from build123d import *

# Parameters (mm, degrees)
FLANGE_PLATE_DEPTH        = 25
BOLT_HOLES_SKETCH_R       = 8
BOLT_HOLES_6X_16_DEPTH    = 25
ANNULAR_RECESS_92_DEPTH   = 15
LUG_HOLES_SKETCH_R        = 7
LUG_HOLES_2X_14_DEPTH     = 111.034083526
KEYED_CENTRE_HUB_40_DEPTH = 15


with BuildPart() as part:
    # Flange Profile Sketch → Flange Plate (new body)
    with BuildSketch(Plane(origin=(0, 0, 0), x_dir=(1, 0, 0), z_dir=(0, 1, 0))):
        with BuildLine():
            ThreePointArc((-14.89981335, 63.269230769), (-32.5, 56.291651246), (-47.342854449, 44.538232258))
            ThreePointArc((-47.342854449, 44.538232258), (-69.282032303, 40), (-62.242667799, 18.730998512))
            ThreePointArc((-62.242667799, 18.730998512), (-65, 0), (-62.242667799, -18.730998512))
            ThreePointArc((-62.242667799, -18.730998512), (-69.282032303, -40), (-47.342854449, -44.538232258))
            ThreePointArc((-47.342854449, -44.538232258), (-32.5, -56.291651246), (-14.89981335, -63.269230769))
            ThreePointArc((-14.89981335, -63.269230769), (0, -80), (14.89981335, -63.269230769))
            ThreePointArc((14.89981335, -63.269230769), (32.5, -56.291651246), (47.342854449, -44.538232258))
            ThreePointArc((47.342854449, -44.538232258), (69.282032303, -40), (62.242667799, -18.730998512))
            ThreePointArc((62.242667799, -18.730998512), (65, 0), (62.242667799, 18.730998512))
            ThreePointArc((62.242667799, 18.730998512), (69.282032303, 40), (47.342854449, 44.538232258))
            ThreePointArc((47.342854449, 44.538232258), (32.5, 56.291651246), (14.89981335, 63.269230769))
            ThreePointArc((14.89981335, 63.269230769), (0, 80), (-14.89981335, 63.269230769))
        make_face()
    extrude(amount=FLANGE_PLATE_DEPTH)

    # Bolt Holes Sketch → Bolt Holes 6xØ16 (cut)
    with BuildSketch(Plane(origin=(0, 25, 0), x_dir=(1, 0, 0), z_dir=(0, 1, 0))):
        with Locations(Location((0, 65, 0), (0, 0, 270))):
            Circle(BOLT_HOLES_SKETCH_R)
        with Locations(Location((56.291651246, 32.5, 0), (0, 0, 270))):
            Circle(BOLT_HOLES_SKETCH_R)
        with Locations(Location((56.291651246, -32.5, 0), (0, 0, 270))):
            Circle(BOLT_HOLES_SKETCH_R)
        with Locations(Location((0, -65, 0), (0, 0, 270))):
            Circle(BOLT_HOLES_SKETCH_R)
        with Locations(Location((-56.291651246, -32.5, 0), (0, 0, 270))):
            Circle(BOLT_HOLES_SKETCH_R)
        with Locations(Location((-56.291651246, 32.5, 0), (0, 0, 270))):
            Circle(BOLT_HOLES_SKETCH_R)
    extrude(amount=-BOLT_HOLES_6X_16_DEPTH, mode=Mode.SUBTRACT)

    # Recess Sketch → Annular Recess Ø92 (cut)
    with BuildSketch(Plane(origin=(0, 25, 0), x_dir=(1, 0, 0), z_dir=(0, 1, 0))):
        with BuildLine():
            ThreePointArc((-43.217391304, -15.756176213), (0, -46), (43.217391304, -15.756176213))
            ThreePointArc((43.217391304, -15.756176213), (30, 0), (43.217391304, 15.756176213))
            ThreePointArc((43.217391304, 15.756176213), (0, 46), (-43.217391304, 15.756176213))
            ThreePointArc((-43.217391304, 15.756176213), (-30, 0), (-43.217391304, -15.756176213))
        make_face()
    extrude(amount=-ANNULAR_RECESS_92_DEPTH, mode=Mode.SUBTRACT)

    # Lug Holes Sketch → Lug Holes 2xØ14 (cut, through all)
    with BuildSketch(Plane(origin=(0, 25, 0), x_dir=(1, 0, 0), z_dir=(0, 1, 0))):
        with Locations(Location((-46, 0, 0), (0, 0, 270))):
            Circle(LUG_HOLES_SKETCH_R)
        with Locations(Location((46, 0, 0), (0, 0, 270))):
            Circle(LUG_HOLES_SKETCH_R)
    extrude(amount=-LUG_HOLES_2X_14_DEPTH, mode=Mode.SUBTRACT)

    # Centre Hub Sketch → Keyed Centre Hub Ø40 (add)
    with BuildSketch(Plane(origin=(0, 10, 0), x_dir=(1, 0, 0), z_dir=(0, 1, 0))):
        with BuildLine():
            Line((17.207997686, -10.192390085), (27.532796297, -16.307824137))
            ThreePointArc((27.532796297, -16.307824137), (22.581559349, -22.673181898), (16.196205348, -27.598603811))
            Line((16.196205348, -27.598603811), (10.122628343, -17.249127382))
            ThreePointArc((10.122628343, -17.249127382), (-0.040491828, -19.99995901), (-10.192390085, -17.207997686))
            Line((-10.192390085, -17.207997686), (-16.307824137, -27.532796297))
            ThreePointArc((-16.307824137, -27.532796297), (-22.673181898, -22.581559349), (-27.598603811, -16.196205348))
            Line((-27.598603811, -16.196205348), (-17.249127382, -10.122628343))
            ThreePointArc((-17.249127382, -10.122628343), (-19.99995901, 0.040491828), (-17.207997686, 10.192390085))
            Line((-17.207997686, 10.192390085), (-27.532796297, 16.307824137))
            ThreePointArc((-27.532796297, 16.307824137), (-22.581559349, 22.673181898), (-16.196205348, 27.598603811))
            Line((-16.196205348, 27.598603811), (-10.122628343, 17.249127382))
            ThreePointArc((-10.122628343, 17.249127382), (0.040491828, 19.99995901), (10.192390085, 17.207997686))
            Line((10.192390085, 17.207997686), (16.307824137, 27.532796297))
            ThreePointArc((16.307824137, 27.532796297), (22.673181898, 22.581559349), (27.598603811, 16.196205348))
            Line((27.598603811, 16.196205348), (17.249127382, 10.122628343))
            ThreePointArc((17.249127382, 10.122628343), (19.99995901, -0.040491828), (17.207997686, -10.192390085))
        make_face()
    extrude(amount=KEYED_CENTRE_HUB_40_DEPTH)


solid = part.part
CAD build for the part. Positions are in the model's coordinates, mm. A direction names the side the tool comes from. Coordinates: 2 decimals unless noted, no trailing zeros. Loops run counter-clockwise (first coordinate to the right, second up) from the corner with the lowest first, then second, coordinate; pieces in that order, holes last. Notation, with made-up numbers: (38, 55.5) -> (60, 55.5) arc R9 cw to (60, 66.5) -> close; hole circle Ø7 at (0, 9). An arc over 180 degrees is marked (long way). One line per item, written item: value.
1. Slice it at C-C on z = 65. Write the cut outline in (x, y), and give its area (3 significant figures).
Answers:
outline: (-15, 0) -> (-8, 0) -> (-8, 25) -> (-15, 25) -> close; (8, 0) -> (15, 0) -> (15, 25) -> (8, 25) -> close
area: 350 mm^2
2. Pull direction X, two halves, no side cores. Call faces 3 (the face through (0, 12, 80)), 4 (the face through (65, 12, 0)), 5 (the face through (69.101, 12.325, 40.305)), 6 (the face through (31, 25, -1)): pulls with the +X half, pulls with the -X half, needs draft (parallel to the pull), parting line crosses it, or undercut.
Answers:
face 3: parting line crosses it
face 4: pulls with the +X half
face 5: undercut
face 6: needs draft
3. Slice it at B-B on x = 0. Write the cut outline in (y, z), and give its area (3 significant figures).
Answers:
outline: (0, -80) -> (25, -80) -> (25, -73) -> (0, -73) -> close; (0, -57) -> (25, -57) -> (25, -46) -> (10, -46) -> (10, -20) -> (25, -20) -> (25, 20) -> (10, 20) -> (10, 46) -> (25, 46) -> (25, 57) -> (0, 57) -> close; (0, 73) -> (25, 73) -> (25, 80) -> (0, 80) -> close
area: 2,420 mm^2
4. Which spindle directions (+Z, -Z, +X, -X, +Y, -Y) get a long thin tool onto all of the face, cutting with end or side? Do faces 1 (the face through (-1, 10, -21)), 2 (the face through (-39.06, 12.68, -0.91)). Say none if no direction does.
Answers:
face 1: +Y
face 2: +Y, -Y
5. Slice it at D-D on y = 2.25. Give the number of separate pieces and of enclosed holes in the cut face, and give its area (3 significant figures).
Answers:
separate pieces: 1
enclosed holes: 8
area: 14,000 mm^2
6. Flat gauge pins, fed straight in: P1, Ø4, axis at x = -40, y = 17, coming from the -Z side; P2, Ø8, axis at y = 13, z = 9, coming from the -X side; P3, Ø11, axis at x = 46, z = 0, coming from the -Y side; P4, Ø1.5, axis at x = 1, y = 15, coming from the -Z side. Where does each tip first touch, or does it go through?
Answers:
P1: stops at z = -52.74
P2: stops at x = -64.81
P3: passes through
P4: stops at z = -80
7. Drill centre lines: line 1 (X direction, y = 19, z = 65); line 2 (Z direction, x = -56, y = 19); line 3 (Z direction, x = 61.5, y = 14.5). Where is each one in solid material? Low to high. Write a range as [from, to].
Answers:
line 1: x = [-15, -8], [8, 15]
line 2: z = [-47.5, -40.49], [-24.51, 24.51], [40.49, 47.5]
line 3: z = [-46.57, -38.57], [-26.43, 26.43], [38.57, 46.57]
8. Slice it at A-A on z = 0. Write the cut outline in (x, y).
Answers:
outline: (-65, 0) -> (-53, 0) -> (-53, 25) -> (-65, 25) -> close; (-39, 0) -> (39, 0) -> (39, 25) -> (30, 25) -> (30, 10) -> (20, 10) -> (20, 25) -> (-20, 25) -> (-20, 10) -> (-30, 10) -> (-30, 25) -> (-39, 25) -> close; (53, 0) -> (65, 0) -> (65, 25) -> (53, 25) -> close
